```python
from build123d import *

# Parameters (mm, degrees)
SKETCH2_RX              = 12.5
SKETCH2_RY              = 7.5
M8_TAPPED_HOLE1_D       = 6.8
M8_TAPPED_HOLE1_DEPTH   = 19.75
M8_TAPPED_HOLE1_TIP     = 2.042926105
SKETCH6_W               = 123
SKETCH6_H               = 44.9
SKETCH6_W_2             = 103
SKETCH6_H_2             = 24.9
CUT_EXTRUDE_THIN1_DEPTH = 107.18262584


with BuildPart() as part:
    # Sweep1: sweep along a path in Sketch3
    with BuildLine(Plane(origin=(0, 0, 0), x_dir=(1, 0, 0), z_dir=(0, 1, 0))) as sweep1_path:
        Line((0, 0), (0, 15))
        ThreePointArc((0, 15), (5.857864376, 29.142135624), (20, 35))
        Line((20, 35), (69, 35))
        ThreePointArc((69, 35), (83.142135624, 29.142135624), (89, 15))
        Line((89, 15), (89, 0))
    # Sketch2 → Sweep1 (sweep)
    with BuildSketch(Plane.XY):
        with Locations(Location((0, 0), (0, 0, 90))):
            Ellipse(SKETCH2_RX, SKETCH2_RY)
    sweep(path=sweep1_path.line)

    # M8 Tapped Hole1
    with Locations(Plane.XY):
        with Locations((0, 0), (89, 0)):
            Hole(M8_TAPPED_HOLE1_D / 2, depth=M8_TAPPED_HOLE1_DEPTH)
            with Locations((0, 0, -(M8_TAPPED_HOLE1_DEPTH + M8_TAPPED_HOLE1_TIP / 2))):  # 118° drill point
                Cone(0, M8_TAPPED_HOLE1_D / 2, M8_TAPPED_HOLE1_TIP, mode=Mode.SUBTRACT)

    # Sketch6 → Cut-Extrude-Thin1 (cut, through all)
    with BuildSketch(Plane.XY):
        with Locations((44.5, 0)):
            Rectangle(SKETCH6_W, SKETCH6_H)
        with Locations((44.5, 0)):
            Rectangle(SKETCH6_W_2, SKETCH6_H_2, mode=Mode.SUBTRACT)
    extrude(amount=-CUT_EXTRUDE_THIN1_DEPTH, mode=Mode.SUBTRACT)


solid = part.part
```
Can you work these out from the model? Positions are in its coordinate system, mm. A direction names the side the tool comes from. Round coordinates to 2 decimals unless told otherwise and drop trailing zeros. Answer in a Markdown table with one row per item.
Item 1: Will these pins go through, and if not, where does the flat tip stop? P1, Ø2, axis at y = -10, z = -22, coming from the +X side; P2, Ø6, axis at x = 89, y = 0, coming from the +Z side; P3, Ø1.5, axis at y = 8.5, z = -23, coming from the +X side; P4, Ø10, axis at x = 7, z = -32, coming from the +Y side.
Answer block:
| item | result |
|---|---|
| P1 | x = 93.27 |
| P2 | z = -19.99 |
| P3 | x = 93.69 |
| P4 | y = 12.45 |
Item 2: On a 3-axis mill with a long thin cutter (end or side, diameter ignored), from which of +Z, -Z, +X, -X, +Y, -Y can I reach the whole of each face in a straight line? I mean faces 4 (the flat face through (2, 3, 0)), 5 (the cylindrical face through (0.74, -3.32, -10.01)). Say none if no direction works.
Answer block:
| item | result |
|---|---|
| face 4 | +Z, +X, -X, +Y, -Y |
| face 5 | +Z |
Item 3: If I drill on probe 1 along X at (y, z) = (0, -6.25); probe 2 along X at (y, z) = (-0.75, -12.5); probe 3 along Y at (x, z) = (0, -5.5), over which ranges is the centre line in solid material (lowest first)?
Answer block:
| item | result |
|---|---|
| probe 1 | -7 to -3.4, 3.4 to 7.5, 81.5 to 85.6, 92.4 to 96 |
| probe 2 | -7 to -3.32, 3.32 to 7.49, 81.51 to 85.68, 92.32 to 96 |
| probe 3 | -12.45 to -3.4, 3.4 to 12.45 |
Item 4: Suppose I cut it at A-A, the plane z = -4. Give the number of separate pieces and of enclosed holes in the cut face, plus the area to 3 significant figures.
Answer block:
| item | result |
|---|---|
| separate pieces | 2 |
| enclosed holes | 2 |
| area | 510 mm² |
Item 5: We'd pull the mould along X, two halves only. Please class faces 1 (the flat face through (-7, 0, -10)), 2 (the flat face through (48, -12.45, -35)), 3 (the cylindrical face through (92.4, 0.1, -10)): released by +X, released by -X, zero draft, split by the parting line, or undercut.
Answer block:
| item | result |
|---|---|
| face 1 | released by -X |
| face 2 | zero draft |
| face 3 | undercut |
